```python
from build123d import *

# Parameters (mm, degrees)
BOSS_EXTRUDE_1_DEPTH = 163


with BuildPart() as part:
    # Sketch 1 → Boss-Extrude 1 (new, symmetric)
    with BuildSketch(Plane.XY):
        with BuildLine():
            Line((0, 32), (-24, 32))
            ThreePointArc((-24, 32), (-29.656854249, 29.656854249), (-32, 24))
            Line((-32, 24), (-32, 0))
            Line((-32, 0), (-32, -24))
            ThreePointArc((-32, -24), (-29.656854249, -29.656854249), (-24, -32))
            Line((-24, -32), (24, -32))
            ThreePointArc((24, -32), (29.656854249, -29.656854249), (32, -24))
            Line((32, -24), (32, 0))
            Line((32, 0), (32, 24))
            ThreePointArc((32, 24), (29.656854249, 29.656854249), (24, 32))
            Line((24, 32), (0, 32))
        make_face()
        with BuildLine():
            Line((0, 28), (-24, 28))
            ThreePointArc((-24, 28), (-26.828427125, 26.828427125), (-28, 24))
            Line((-28, 24), (-28, 0))
            Line((-28, 0), (-28, -24))
            ThreePointArc((-28, -24), (-26.828427125, -26.828427125), (-24, -28))
            Line((-24, -28), (24, -28))
            ThreePointArc((24, -28), (26.828427125, -26.828427125), (28, -24))
            Line((28, -24), (28, 0))
            Line((28, 0), (28, 24))
            ThreePointArc((28, 24), (26.828427125, 26.828427125), (24, 28))
            Line((24, 28), (0, 28))
        make_face(mode=Mode.SUBTRACT)
    extrude(amount=BOSS_EXTRUDE_1_DEPTH, both=True)


solid = part.part
```
Read the model definition and answer for the solid it produces. Units are mm, in the model's axes. A direction names the side the tool comes from. Give positions to 0.01 mm unless a question says otherwise; leave off trailing zeros. Order: outer loops, then holes, each group sorted by start corner. A loop starts at its lowest first (then second) coordinate and runs counter-clockwise, first axis right, second up.
(1) Straight lines are drawn through the part: L1, parallel to X at y = -2.5, z = 60.5; L2, parallel to Y at x = 25, z = 92. For each, find the intervals that lie inside material, in ascending order.
(2) For faces 1 (the flat face through (0, 28, 2)), 2 (the flat face through (32, 0, 2)), determine the directions among +Z, -Z, +X, -X, +Y, -Y from which every point of the face is accessible in a straight line to the end or side of a thin tool.
(3) Find section C-C (z = 50.5). Give the vertices of the cut face in (x, y).
(4) For a pull along X with two mould halves and no side action, classify faces 3 (the flat face through (-32, 0, 2)), 4 (the flat face through (0, 32, 2)), 5 (the flat face through (0, -28, 2)), 6 (the cylindrical face through (29.719, 29.594, 2.282)) as released by +X, released by -X, zero draft, split by the parting line, or undercut.
(5) Find section A-A (x = 1.5). Give the vertices of the cut face in (y, z), plus the area to 3 significant figures.
Result sheet:
1. L1: x = -32 to -28, 28 to 32
1. L2: y = -31.94 to -27.87, 27.87 to 31.94
2. face 1: +Z, -Z
2. face 2: +Z, -Z, +X, +Y, -Y
3. outline: (-32, -24) arc R8 ccw to (-24, -32) - (24, -32) arc R8 ccw to (32, -24) - (32, 24) arc R8 ccw to (24, 32) - (-24, 32) arc R8 ccw to (-32, 24) - close; hole (-28, -24) arc R4 ccw to (-24, -28) - (24, -28) arc R4 ccw to (28, -24) - (28, 24) arc R4 ccw to (24, 28) - (-24, 28) arc R4 ccw to (-28, 24) - close
4. face 3: released by -X
4. face 4: zero draft
4. face 5: undercut
4. face 6: released by +X
5. outline: (-32, -163) - (-28, -163) - (-28, 163) - (-32, 163) - close; (28, -163) - (32, -163) - (32, 163) - (28, 163) - close
5. area: 2,610 mm2
